Check sheet for the modelled part. Datum: model origin and axes. Units: mm. Round coordinates to 2 decimals unless told otherwise and drop trailing zeros. Write each loop counter-clockwise with the first axis right and the second up, starting at its lowest first coordinate (ties: lowest second). Pieces come first, ordered by that corner, then holes.
from build123d import *

# Parameters (mm, degrees)
SKETCH1_R               = 5
BOSS_EXTRUDE1_DEPTH     = 23
SKETCH2_R               = 4
BOSS_EXTRUDE2_DEPTH     = 18
CHAMFER1_SIZE           = 0.5
CUT_EXTRUDE1_DEPTH      = 25.062418831
CUT_EXTRUDE1_DEPTH_BACK = 25.062418831
SKETCH3_R               = 3


with BuildPart() as part:
    # Sketch1 → Boss-Extrude1 (new body)
    with BuildSketch(Plane.XY):
        Circle(SKETCH1_R)
    extrude(amount=BOSS_EXTRUDE1_DEPTH)

    # Sketch2 → Boss-Extrude2 (add)
    with BuildSketch(Plane(origin=(0, 0, 0), x_dir=(-1, 0, 0), z_dir=(0, 0, -1))):
        Circle(SKETCH2_R)
    extrude(amount=BOSS_EXTRUDE2_DEPTH)

    # Chamfer1
    chamfer1_edges = [part.edges().sort_by_distance(p)[0] for p in [
        (-5, 0, 23),
        (4, 0, -18),
    ]]
    chamfer(chamfer1_edges, length=CHAMFER1_SIZE)

    # Sketch3 → Cut-Extrude1 (cut, two sides: drawn at the far end of the back side and taken through both)
    with BuildSketch(Plane(origin=(0, 0, 0), x_dir=(1, 0, 0), z_dir=(0, 1, 0)).offset(-CUT_EXTRUDE1_DEPTH_BACK)):
        with Locations(Location((0, -18, 0), (0, 0, 270))):
            Circle(SKETCH3_R)
    extrude(amount=CUT_EXTRUDE1_DEPTH + CUT_EXTRUDE1_DEPTH_BACK, mode=Mode.SUBTRACT)


solid = part.part
1. Sectioned sample at A-A, the plane x = 0. Enter the section's corners in (y, z), plus the area to 4 significant figures.
2. Scan lines: line 1 along Z through (x, y) = (0, 0.5); line 2 along X through (y, z) = (3, 18); line 3 along X through (y, z) = (-3, 4). Record each from-to range of solid material in increasing order.
3. Sectioned sample at C-C, the plane z = -1. Enter the section's corners in (x, y).
4. Go/stop test with flat-tipped pins: pin 1 (6 mm diameter, centred on x = -3.5, z = 17, fed in from +Y); pin 2 (4 mm diameter, centred on y = -0.5, z = -11.5, fed in from +X). Record where each tip stops, or that it passes through.
5. Release check for a two-part mould opening along Z. For faces 1 (the cylindrical face through (0, 0, 15)), 2 (the flat face through (0, 0, -18)), 3 (the flat face through (0, 0, 23)), 4 (the cylindrical face through (0.867, -3.905, -8.628)) record: released by +Z, released by -Z, zero draft, split by the parting line, or undercut.
6. Sectioned sample at B-B, the plane y = 0. Enter the section's corners in (x, z), plus the area to 3 significant figures.
7. Sectioned sample at D-D, the plane z = 6. Enter the section's corners in (x, y), plus the area to 3 significant figures.
Computed values:
1. outline: (-5, 0) - (-4, 0) - (-4, -17.5) - (-3.5, -18) - (3.5, -18) - (4, -17.5) - (4, 0) - (5, 0) - (5, 15) - (-5, 15) - close; (-5, 21) - (5, 21) - (5, 22.5) - (4.5, 23) - (-4.5, 23) - (-5, 22.5) - close
1. area: 313.5 mm2
2. line 1: z = -18 to 15, 21 to 23
2. line 2: x = -4 to -3, 3 to 4
2. line 3: x = -4 to 4
3. outline: circle Ø8 at (0, 0)
4. pin 1: stops at y = 4.88
4. pin 2: stops at x = 4
5. face 1: undercut
5. face 2: released by -Z
5. face 3: released by +Z
5. face 4: zero draft
6. outline: (-5, 0) - (-4, 0) - (-4, -17.5) - (-3.5, -18) - (3.5, -18) - (4, -17.5) - (4, 0) - (5, 0) - (5, 22.5) - (4.5, 23) - (-4.5, 23) - (-5, 22.5) - close; hole circle Ø6 at (0, 18)
6. area: 345 mm2
7. outline: circle Ø10 at (0, 0)
7. area: 78.5 mm2
